```python
from build123d import *

# Parameters (mm, degrees)
SKETCH_1_W             = 80
SKETCH_1_H             = 94.5
EXTRUDE_1_DEPTH        = 14
HOLE_WIZARD_M6_1_D     = 5
HOLE_WIZARD_M6_1_DEPTH = 17
HOLE_WIZARD_M6_1_TIP   = 1.502151548
HOLE_WIZARD_M6_2_D     = 5
HOLE_WIZARD_M6_2_DEPTH = 17
HOLE_WIZARD_M6_2_TIP   = 1.502151548


with BuildPart() as part:
    # 草图1 → 凸台-拉伸1 (new body)
    with BuildSketch(Plane.XY):
        Rectangle(SKETCH_1_W, SKETCH_1_H)
    extrude(amount=EXTRUDE_1_DEPTH)

    # M6 螺纹孔1
    with Locations(Plane(origin=(0, -47.25, 0), x_dir=(-1, 0, 0), z_dir=(0, -1, 0))):
        with Locations((-21, -7), (21, -7)):
            Hole(HOLE_WIZARD_M6_1_D / 2, depth=HOLE_WIZARD_M6_1_DEPTH)
            with Locations((0, 0, -(HOLE_WIZARD_M6_1_DEPTH + HOLE_WIZARD_M6_1_TIP / 2))):  # 118° drill point
                Cone(0, HOLE_WIZARD_M6_1_D / 2, HOLE_WIZARD_M6_1_TIP, mode=Mode.SUBTRACT)

    # M6 螺纹孔2
    with Locations(Plane(origin=(0, 47.25, 0), x_dir=(1, 0, 0), z_dir=(0, 1, 0))):
        with Locations((33, -7), (-33, -7)):
            Hole(HOLE_WIZARD_M6_2_D / 2, depth=HOLE_WIZARD_M6_2_DEPTH)
            with Locations((0, 0, -(HOLE_WIZARD_M6_2_DEPTH + HOLE_WIZARD_M6_2_TIP / 2))):  # 118° drill point
                Cone(0, HOLE_WIZARD_M6_2_D / 2, HOLE_WIZARD_M6_2_TIP, mode=Mode.SUBTRACT)


solid = part.part
```
Verification items for the finished model (mm, model axes). A direction names the side the tool comes from. Coordinates: 2 decimals unless noted, no trailing zeros. Answer in a Markdown table with one row per item. Add a question column.
1. Draft check along X on faces 4 (the face through (-1, 1, 0)), 5 (the face through (-40, -1, 7)), 6 (the face through (33.23, 29.01, 6.63)). Enter one of: +X half, -X half, draft (parallel to the pull), parting line (faces both ways), or undercut.
2. Access from +Z, -Z, +X, -X, +Y, -Y to the whole of each face (thin tool, end or side, straight path). Record for faces 1 (the face through (-35.31, 38.63, 7.96)), 2 (the face through (-23.5, -38.6, 6.9)), 3 (the face through (-1, 47.25, 7)).
3. Depth check by flat-ended pin: P1, Ø4, axis at x = -33, z = 7, coming from the +Y side. Enter the tip coordinate at first touch or a pass-through.
4. Material ranges on probe 1 along Z at (x, y) = (-33, 43.5), recorded low to high. Write a range as [from, to].
Derived:
| question | item | result |
|---|---|---|
| 1 | face 4 | draft |
| 1 | face 5 | -X half |
| 1 | face 6 | undercut |
| 2 | face 1 | +Y |
| 2 | face 2 | -Y |
| 2 | face 3 | +Z, -Z, +X, -X, +Y |
| 3 | P1 | stops at y = 29.95 |
| 4 | probe 1 | z = [0, 4.5], [9.5, 14] |
